from build123d import *

# Parameters (mm, degrees)
SKETCH1_R             = 3
BOSS_EXTRUDE1_DEPTH   = 3
SKETCH2_R             = 6
BOSS_EXTRUDE2_DEPTH   = 2.5
BOSS_EXTRUDE3_START   = 2.5
SKETCH3_R             = 6
BOSS_EXTRUDE3_DEPTH   = 2.5
SKETCH4_R             = 4.25
BOSS_EXTRUDE4_DEPTH   = 15
SKETCH5_R             = 1
CUT_EXTRUDE1_DEPTH    = 7
M5_TAPPED_HOLE1_D     = 4.2
M5_TAPPED_HOLE1_DEPTH = 12
M5_TAPPED_HOLE1_TIP   = 1.2618073
SKETCH7_W             = 2.207825045
SKETCH7_H             = 11.152764798
CUT_EXTRUDE2_DEPTH    = 5


with BuildPart() as part:
    # Sketch1 → Boss-Extrude1 (new body)
    with BuildSketch(Plane(origin=(0, 0, 0), x_dir=(1, 0, 0), z_dir=(0, 1, 0))):
        with Locations(Location((0, 0, 0), (0, 0, 270))):
            Circle(SKETCH1_R)
    extrude(amount=BOSS_EXTRUDE1_DEPTH)

    # Sketch2 → Boss-Extrude2 (add)
    with BuildSketch(Plane(origin=(0, 3, 0), x_dir=(1, 0, 0), z_dir=(0, 1, 0))):
        with Locations(Location((0, 0, 0), (0, 0, 270))):
            Circle(SKETCH2_R)
    extrude(amount=BOSS_EXTRUDE2_DEPTH)

    # Sketch3 → Boss-Extrude3 (add)
    with BuildSketch(Plane.XZ.offset(BOSS_EXTRUDE3_START)):
        with Locations(Location((0, 0, 0), (0, 0, 90))):
            Circle(SKETCH3_R)
    extrude(amount=-BOSS_EXTRUDE3_DEPTH)

    # Sketch4 → Boss-Extrude4 (add)
    with BuildSketch(Plane.XZ.offset(2.5)):
        with Locations(Location((0, 0, 0), (0, 0, 270))):
            Circle(SKETCH4_R)
    extrude(amount=BOSS_EXTRUDE4_DEPTH)

    # Sketch5 → Cut-Extrude1 (cut)
    with BuildSketch(Plane.XZ.offset(17.5)):
        with Locations(Location((0, 0, 0), (0, 0, 270))):
            Circle(SKETCH5_R)
    extrude(amount=-CUT_EXTRUDE1_DEPTH, mode=Mode.SUBTRACT)

    # M5 Tapped Hole1
    with Locations(Plane(origin=(0, -17.5, 0), x_dir=(0, 0, -1), z_dir=(0, -1, 0))):
        with Locations((0, 0)):
            Hole(M5_TAPPED_HOLE1_D / 2, depth=M5_TAPPED_HOLE1_DEPTH)
            with Locations((0, 0, -(M5_TAPPED_HOLE1_DEPTH + M5_TAPPED_HOLE1_TIP / 2))):  # 118° drill point
                Cone(0, M5_TAPPED_HOLE1_D / 2, M5_TAPPED_HOLE1_TIP, mode=Mode.SUBTRACT)

    # Sketch7 → Cut-Extrude2 (cut, symmetric)
    with BuildSketch(Plane(origin=(0, 0, 0), x_dir=(0, 0, -1), z_dir=(1, 0, 0))):
        with Locations((4.853912523, -11.923617601)):
            Rectangle(SKETCH7_W, SKETCH7_H)
        with Locations((-4.853912523, -11.923617601)):
            Rectangle(SKETCH7_W, SKETCH7_H)
    extrude(amount=CUT_EXTRUDE2_DEPTH, both=True, mode=Mode.SUBTRACT)


solid = part.part
For this review, take the finished solid that the model builds, in its own axes (mm). A direction names the side the tool comes from. Give positions to 0.01 mm unless a question says otherwise; leave off trailing zeros. Loops run counter-clockwise (first coordinate to the right, second up) from the corner with the lowest first, then second, coordinate; pieces in that order, holes last. Notation, with made-up numbers: M 30,-5.5 L 61,-5.5 A9 cw 61,10.5 Z; hole C 75,6.5 d3. An arc over 180 degrees is marked long. Put each result on its own line as item: value. Start each with the question number.
(1) Add section D-D, the plane y = -1. Write out the cut boundary in (x, z), then the cut area to 3 significant figures.
(2) Add section B-B, the plane y = -9.75. Write out the cut boundary in (x, z).
(3) Wall thickness on L1, parallel to Y at x = 3.5, z = 1.75; L2, parallel to Y at x = 5, z = -0.5; L3, parallel to Z at x = 0, y = -9.5: over which ranges is each line inside the solid? List them lowest first.
(4) Machinability: for faces 1 (the cylindrical face through (0.631, -11.416, 2.003)), 2 (the flat face through (-3, 0, 1)), 3 (the flat face through (0, -12, 3.75)), 4 (the flat face through (0, -12, -3.75)), which of the approach directions +Z, -Z, +X, -X, +Y, -Y give a long, thin tool a straight path to every point of the face, cutting with its end or side? Answer none if there is none.
(5) For pin 1 (3.5 mm diameter, centred on x = -0.5, z = 2, fed in from -Y); pin 2 (4 mm diameter, centred on y = -9.5, z = 4.5, fed in from +X); pin 3 (3 mm diameter, centred on x = 0, y = -13, fed in from +Z); pin 4 (1.5 mm diameter, centred on x = 4.5, y = -13.5, fed in from -Z), all flat-tipped, find the tip position at first contact; note any pin that passes through.
(6) The part is to be moulded in two halves that separate along X. For faces 5 (the conical face through (0.11, -4.46, -0.35)), 6 (the flat face through (4, -2.5, 3)), 7 (the cylindrical face through (0.9, 1.48, 2.86)), say which applies: +X half, -X half, draft (parallel to the pull), parting line (faces both ways), or undercut.
(7) Add section C-C, the plane x = -5. Write out the cut boundary in (y, z), then the cut area to 3 significant figures.
(8) Add section A-A, the plane x = 3.5. Write out the cut boundary in (y, z), then the cut area to 3 significant figures.
Result:
1. outline: C 0,0 d12
1. area: 113 mm^2
2. outline: M -2,-3.75 L 2,-3.75 A4.25 ccw 2,3.75 L -2,3.75 A4.25 ccw Z; hole C 0,0 d4.2
3. L1: y = -17.5 to 0, 3 to 5.5
3. L2: y = -2.5 to 0, 3 to 5.5
3. L3: z = -3.75 to -2.1, 2.1 to 3.75
4. face 1: -Y
4. face 2: none
4. face 3: +Z, +X, -X, -Y
4. face 4: -Z, +X, -X, -Y
5. pin 1: stops at y = -17.5
5. pin 2: stops at x = 3.44
5. pin 3: stops at z = 3.75
5. pin 4: stops at z = -2
6. face 5: undercut
6. face 6: draft
6. face 7: parting line
7. outline: M -2.5,-3.32 L 0,-3.32 L 0,3.32 L -2.5,3.32 Z; M 3,-3.32 L 5.5,-3.32 L 5.5,3.32 L 3,3.32 Z
7. area: 33.2 mm^2
8. outline: M -17.5,-2.41 L -2.5,-2.41 L -2.5,-4.87 L 0,-4.87 L 0,4.87 L -2.5,4.87 L -2.5,2.41 L -17.5,2.41 Z; M 3,-4.87 L 5.5,-4.87 L 5.5,4.87 L 3,4.87 Z
8. area: 121 mm^2
